from build123d import *

# Parameters (mm, degrees)
SKETCH_1_W                  = 70
SKETCH_1_H                  = 57
EXTRUDE_1_DEPTH             = 10
SKETCH_2_W                  = 70
SKETCH_2_H                  = 10
EXTRUDE_2_DEPTH             = 15
CHAMFER_1_SIZE              = 3
HOLE_WIZARD_M4_1_D          = 3.3
HOLE_WIZARD_M4_1_DEPTH      = 10.1
HOLE_WIZARD_M4_1_TIP        = 0.991420021
HOLE_WIZARD_5_5_5_5_1_D     = 5.5
HOLE_WIZARD_5_5_5_5_1_DEPTH = 10.1
HOLE_WIZARD_5_5_5_5_1_TIP   = 1.652366702


with BuildPart() as part:
    # 草图1 → 凸台-拉伸1 (new body)
    with BuildSketch(Plane(origin=(0, 0, 0), x_dir=(1, 0, 0), z_dir=(0, 1, 0))):
        Rectangle(SKETCH_1_W, SKETCH_1_H)
    extrude(amount=EXTRUDE_1_DEPTH)

    # 草图2 → 凸台-拉伸2 (add)
    with BuildSketch(Plane.XZ):
        with Locations((0, -23.5)):
            Rectangle(SKETCH_2_W, SKETCH_2_H)
    extrude(amount=EXTRUDE_2_DEPTH)

    # 倒角1
    chamfer_1_edges = [part.edges().sort_by_distance(p)[0] for p in [
        (35, -15, -23.5),
        (-35, -15, -23.5),
        (35, 5, 28.5),
        (-35, 5, 28.5),
    ]]
    chamfer(chamfer_1_edges, length=CHAMFER_1_SIZE)

    # M4 螺纹孔1
    with Locations(Plane(origin=(0, 10, 0), x_dir=(1, 0, 0), z_dir=(0, 1, 0))):
        with Locations((32, -3.5), (-18, -3.5), (7, -3.5)):
            Hole(HOLE_WIZARD_M4_1_D / 2, depth=HOLE_WIZARD_M4_1_DEPTH)
            with Locations((0, 0, -(HOLE_WIZARD_M4_1_DEPTH + HOLE_WIZARD_M4_1_TIP / 2))):  # 118° drill point
                Cone(0, HOLE_WIZARD_M4_1_D / 2, HOLE_WIZARD_M4_1_TIP, mode=Mode.SUBTRACT)

    # Ø5.5 (5.5) 直径孔1
    with Locations(Plane.XY.offset(-18.5)):
        with Locations((-15, -7.5), (-30, -7.5)):
            Hole(HOLE_WIZARD_5_5_5_5_1_D / 2, depth=HOLE_WIZARD_5_5_5_5_1_DEPTH)
            with Locations((0, 0, -(HOLE_WIZARD_5_5_5_5_1_DEPTH + HOLE_WIZARD_5_5_5_5_1_TIP / 2))):  # 118° drill point
                Cone(0, HOLE_WIZARD_5_5_5_5_1_D / 2, HOLE_WIZARD_5_5_5_5_1_TIP, mode=Mode.SUBTRACT)


solid = part.part
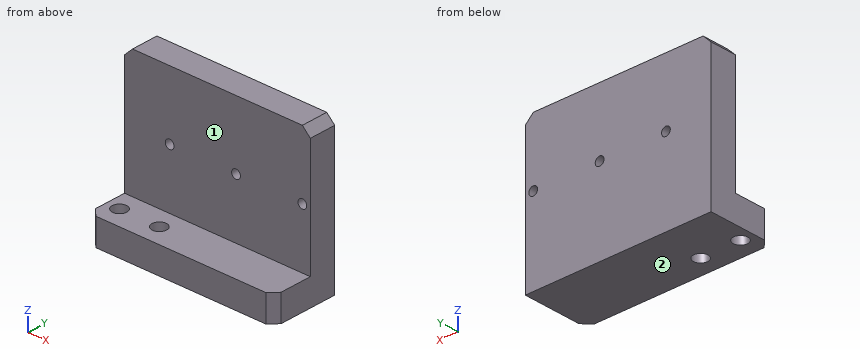
Build history of the part. All positions in model axes, mm. Face numbers are marked on the shaded views. A direction names the side the tool comes from. Round coordinates to 2 decimals unless told otherwise and drop trailing zeros. Loops run counter-clockwise (first coordinate to the right, second up) from the corner with the lowest first, then second, coordinate; pieces in that order, holes last. Notation, with made-up numbers: (87, -25) -> (145, -25) arc R34 cw to (145, 9) -> close; hole circle Ø8 at (41.25, 39). An arc over 180 degrees is marked (long way). Answer in a Markdown table with one row per item.
Item 1: Saw through at D-D (x = -15). Write the cut outline in (y, z), and give its area (3 significant figures).
Answers below:
| item | result |
|---|---|
| outline | (-15, -28.5) -> (-10.25, -28.5) -> (-10.25, -18.5) -> (-15, -18.5) -> close; (-4.75, -28.5) -> (10, -28.5) -> (10, 28.5) -> (0, 28.5) -> (0, -18.5) -> (-4.75, -18.5) -> close |
| area | 665 mm² |
Item 2: Saw through at C-C (z = 3.5). Write the cut outline in (x, y).
Answers below:
| item | result |
|---|---|
| outline | (-35, 0) -> (-19.65, 0) -> (-19.65, 10) -> (-35, 10) -> close; (-16.35, 0) -> (5.35, 0) -> (5.35, 10) -> (-16.35, 10) -> close; (8.65, 0) -> (30.35, 0) -> (30.35, 10) -> (8.65, 10) -> close; (33.65, 0) -> (35, 0) -> (35, 10) -> (33.65, 10) -> close |
Item 3: Pin check, flat tips, straight feed: pin 1 (9 mm diameter, centred on x = -30, y = -7.5, fed in from +Z); pin 2 (23.5 mm diameter, centred on x = -2.5, z = 9, fed in from -Y). Stop position of each tip, or through.
Answers below:
| item | result |
|---|---|
| pin 1 | stops at z = -18.5 |
| pin 2 | stops at y = 0 |
Item 4: Saw through at B-B (y = -7.5). Write the cut outline in (x, z), and give its area (3 significant figures).
Answers below:
| item | result |
|---|---|
| outline | (-35, -28.5) -> (-32.75, -28.5) -> (-32.75, -18.5) -> (-35, -18.5) -> close; (-27.25, -28.5) -> (-17.75, -28.5) -> (-17.75, -18.5) -> (-27.25, -18.5) -> close; (-12.25, -28.5) -> (35, -28.5) -> (35, -18.5) -> (-12.25, -18.5) -> close |
| area | 590 mm² |
Item 5: Which spindle directions (+Z, -Z, +X, -X, +Y, -Y) get a long thin tool onto all of the face, cutting with end or side? Do the marked faces 1 and 2. Say none if no direction does.
Answers below:
| item | result |
|---|---|
| face 1 | +Z, +X, -X, -Y |
| face 2 | -Z, +X, -X, +Y, -Y |
Item 6: Drill centre lines: L1, parallel to Z at x = 32, y = 9.25; L2, parallel to Y at x = 15.5, z = -12; L3, parallel to Y at x = -15, z = -20. Where is each one in solid material? Low to high. Write a range as [from, to].
Answers below:
| item | result |
|---|---|
| L1 | z = [-28.5, 1.85], [5.15, 28.5] |
| L2 | y = [0, 10] |
| L3 | y = [-15, -10.25], [-4.75, 10] |
Item 7: Saw through at A-A (x = 7). Write the cut outline in (y, z).
Answers below:
| item | result |
|---|---|
| outline | (-15, -28.5) -> (10, -28.5) -> (10, 1.85) -> (0, 1.85) -> (0, -18.5) -> (-15, -18.5) -> close; (0, 5.15) -> (10, 5.15) -> (10, 28.5) -> (0, 28.5) -> close |
